Could you check a few things on this drawing? It's one solid part, dimensions in mm from its lowest x, y, z. Coordinates: 2 decimals unless noted, no trailing zeros. Write each loop counter-clockwise with the first axis right and the second up, starting at its lowest first coordinate (ties: lowest second). Pieces come first, ordered by that corner, then holes.
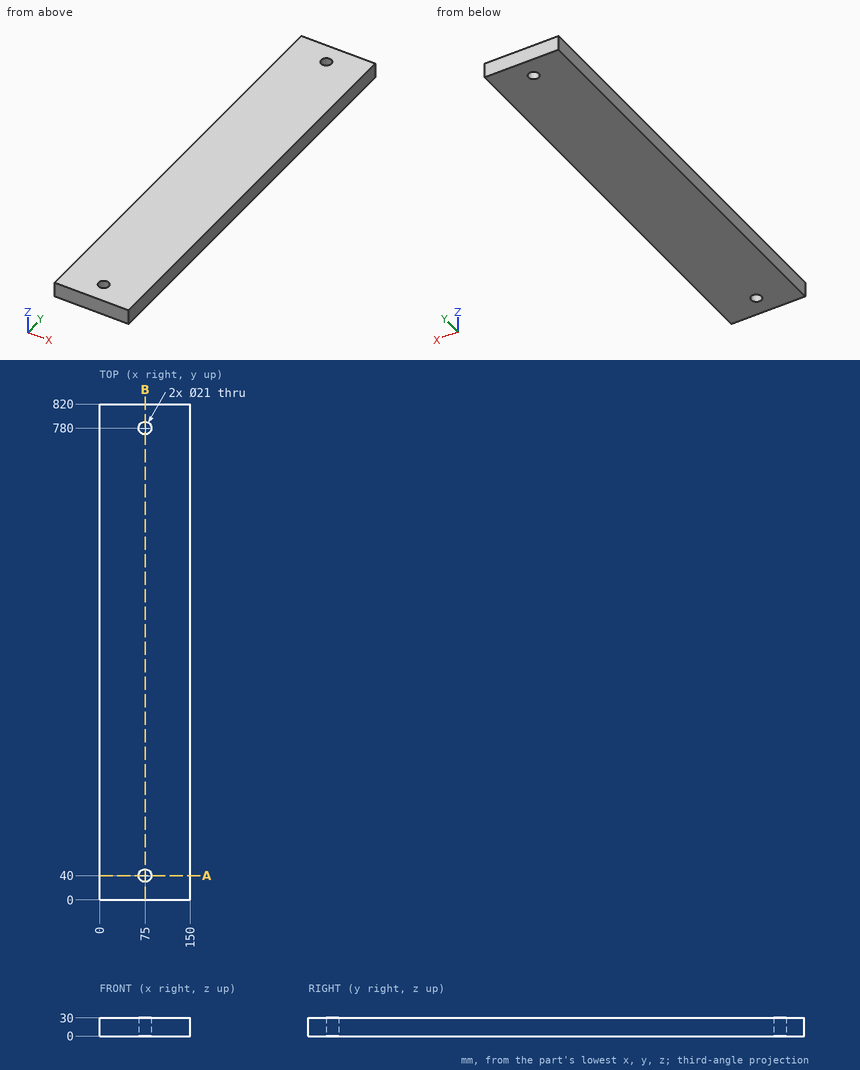
1) Will this pin go through, and if not, where does the flat tip stop? pin 1 (12.5 mm diameter, centred on x = 75, y = 40, fed in from -Z).
Values follow:
pin 1: passes through
2) I need wall thicknesses on probe 1 along Y at (x, z) = (75, 15.25); probe 2 along Y at (x, z) = (73.5, 2.75); probe 3 along X at (y, z) = (780, 9.25). Which ranges of each line are inside material? Lowest first, please.
Values follow:
probe 1: y = 0 to 29.5, 50.5 to 769.5, 790.5 to 820
probe 2: y = 0 to 29.61, 50.39 to 769.61, 790.39 to 820
probe 3: x = 0 to 64.5, 85.5 to 150
3) Imagine slicing it at A-A on y = 40. Please give me the cut outline in (x, z).
Values follow:
outline: (0, 0) - (64.5, 0) - (64.5, 30) - (0, 30) - close; (85.5, 0) - (150, 0) - (150, 30) - (85.5, 30) - close
4) Imagine slicing it at B-B on x = 75. Please give me the cut outline in (y, z).
Values follow:
outline: (0, 0) - (29.5, 0) - (29.5, 30) - (0, 30) - close; (50.5, 0) - (769.5, 0) - (769.5, 30) - (50.5, 30) - close; (790.5, 0) - (820, 0) - (820, 30) - (790.5, 30) - close
